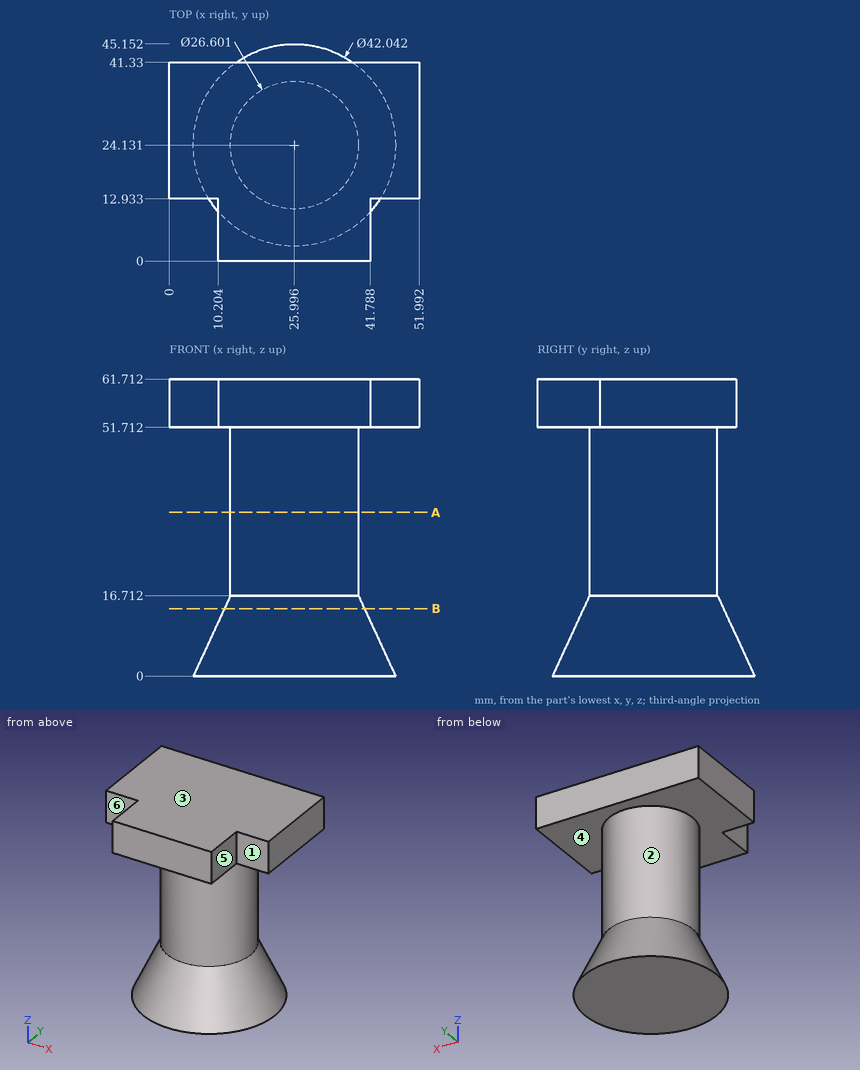
Geometry: see drawing. Coordinates: mm, zero at the bounding-box minimum. A direction names the side the tool comes from. Give positions to 0.01 mm unless a question says otherwise; leave off trailing zeros. Order: outer loops, then holes, each group sorted by start corner. A loop starts at its lowest first (then second) coordinate and runs counter-clockwise, first axis right, second up. Notation, with made-up numbers: (-8.5, -8) - (-3.5, -8) arc R27 cw to (-3.5, 15) - close; hole circle Ø7 at (67.25, -14.5). An arc over 180 degrees is marked (long way). One line per item, written item: value.
1. Line query: probe 1 along Z at (x, y) = (40, 2); probe 2 along X at (y, z) = (24, 38.5); probe 3 along Y at (x, z) = (18, 55.5). Output: solid intervals per line, ascending.
Determined:
probe 1: 51.71 to 61.71
probe 2: 12.7 to 39.3
probe 3: 0 to 41.33
2. Pin query (flat end, axial travel): pin 1 Ø11 at (y, z) = (4, 57) entering from -X; pin 2 Ø8 at (x, z) = (42, 55) entering from +Y; pin 3 Ø5 at (x, z) = (3, 58.5) entering from -Y. Return the tip coordinate at first contact, or that it passes through.
Determined:
pin 1: x = 10.2
pin 2: y = 41.33
pin 3: y = 12.93
3. Cut plane B-B, the plane z = 14. Output: boundary loops of the cut face in (x, y).
Determined:
outline: circle Ø29.11 at (26, 24.13)
4. Reachability of the marked faces 4, 5 and 6 from +Z, -Z, +X, -X, +Y, -Y: full face, straight path, thin tool, end or side. Return the list, or none.
Determined:
face 4: none
face 5: +Z, +X, -Y
face 6: +Z, -X, -Y
5. Draft query along Z for the marked faces 1, 2 and 3. Return one class per face: released by +Z, released by -Z, zero draft, split by the parting line, or undercut.
Determined:
face 1: zero draft
face 2: undercut
face 3: released by +Z
6. Cut plane A-A, the plane z = 34. Output: boundary loops of the cut face in (x, y), and give its area (3 significant figures).
Determined:
outline: circle Ø26.6 at (26, 24.13)
area: 556 mm2
